Could you check a few things on this model? Use its own coordinates, in mm. A direction names the side the tool comes from. Give positions to 0.01 mm unless a question says otherwise; leave off trailing zeros. Loops run counter-clockwise (first coordinate to the right, second up) from the corner with the lowest first, then second, coordinate; pieces in that order, holes last. Notation, with made-up numbers: (89, -16) - (148, -16) arc R29 cw to (148, 8) - close; hole circle Ø4 at (-34.75, 31.5). An arc over 180 degrees is marked (long way). One line per item, written item: value. Start each with the question number.
Q1. I want a section at B-B (z = -75). Count the separate pieces of the cut face and the enclosed holes in it, then the cut area to 4 significant figures.
Q2. If I drill on line 1 (Z direction, x = -70, y = -0.85); line 2 (Z direction, x = 31, y = -1.4); line 3 (X direction, y = -1.8, z = 147.5), over which ranges is the centre line in solid material (lowest first)? Write a range as from..to.
Q3. For faces 5 (the face through (77.15, -0.04, 93.01)), 6 (the face through (-2, 2.5, -59)), which set-ups out of +Z, -Z, +X, -X, +Y, -Y let a thin tool reach every point of the face, with its end or its side?
Q4. If we mould it in two halves opening along Z, with no side actions, what happens to faces 1 (the face through (42.932, 0.035, -76.041)), 2 (the face through (-2, -2.5, -59)), 3 (the face through (-111.867, -0.035, -244.587)), 4 (the face through (-111.867, 0.035, 244.587))? For each: released by +Z, released by -Z, zero draft, split by the parting line, or undercut.
Q5. I want a section at A-A (z = 141). Please give me the cut outline in (x, y).
Q6. I'm going to push flat-ended pins straight in: P1, Ø3, axis at x = -35, z = 12, coming from the -Y side; P2, Ø4, axis at x = -35, z = -63, coming from the +Y side. Where does each tip first touch, or does it pass through?
```python
from build123d import *

# Parameters (mm, degrees)
SKETCH1_W            = 234
SKETCH1_H            = 500
BOSS_EXTRUDE1_DEPTH  = 2.5
M4_CLEARANCE_HOLE1_D = 4.8
FILLET1_R            = 18
M4_TAPPED_HOLE7_D    = 3.3
SKETCH4_R            = 14.75
SKETCH4_R_2          = 8
CUT_EXTRUDE6_DEPTH   = 277.068831997
M4_TAPPED_HOLE3_D    = 3.3
SKETCH9_R            = 14.75
CUT_EXTRUDE3_DEPTH   = 277.068831997
M4_TAPPED_HOLE4_D    = 3.3
SKETCH12_W           = 160
SKETCH12_H           = 120
CUT_EXTRUDE4_DEPTH   = 277.068831997
FILLET2_R            = 10


with BuildPart() as part:
    # Sketch1 → Boss-Extrude1 (new, symmetric)
    with BuildSketch(Plane(origin=(0, 0, 0), x_dir=(1, 0, 0), z_dir=(0, 1, 0))):
        Rectangle(SKETCH1_W, SKETCH1_H)
    extrude(amount=BOSS_EXTRUDE1_DEPTH, both=True)

    # M4 Clearance Hole1 (through all)
    with Locations(Plane(origin=(-75, 2.5, -242.5), x_dir=(0, 0, 1), z_dir=(0, 1, 0))):
        with Locations((0, 0), (0, 150), (67.5, 184.5), (67.5, -34.5), (242.5, 184.5), (242.5, -34.5), (417.5, -34.5), (417.5, 184.5), (485, 0), (485, 150)):
            Hole(M4_CLEARANCE_HOLE1_D / 2)

    # Fillet1
    fillet1_edges = [part.edges().sort_by_distance(p)[0] for p in [
        (117, 0, 250),
        (-117, 0, 250),
        (-117, 0, -250),
        (117, 0, -250),
    ]]
    fillet(fillet1_edges, radius=FILLET1_R)

    # M4 Tapped Hole7 (through all)
    with Locations(Plane(origin=(-85, 2.5, -87), x_dir=(0, 0, 1), z_dir=(0, 1, 0))):
        with Locations((0, 0), (24, 0), (24, 25), (0, 25), (0, 50), (24, 50), (-6, 85), (30, 85), (0, 120), (24, 120), (0, 145), (24, 145), (0, 170), (24, 170), (75, 120), (99, 120), (75, 50), (99, 50)):
            Hole(M4_TAPPED_HOLE7_D / 2)

    # Sketch4 → Cut-Extrude6 (cut, through all)
    with BuildSketch(Plane(origin=(0, 2.5, 0), x_dir=(1, 0, 0), z_dir=(0, 1, 0))):
        with Locations(Location((0, 75, 0), (0, 0, 270))):
            Circle(SKETCH4_R)
        with Locations(Location((-35, 75, 0), (0, 0, 270))):
            Circle(SKETCH4_R_2)
        with Locations(Location((35, 75, 0), (0, 0, 270))):
            Circle(SKETCH4_R_2)
        with Locations(Location((-60, 75, 0), (0, 0, 270))):
            Circle(SKETCH4_R_2)
        with Locations(Location((-85, 75, 0), (0, 0, 270))):
            Circle(SKETCH4_R_2)
        with Locations(Location((60, 75, 0), (0, 0, 270))):
            Circle(SKETCH4_R_2)
        with Locations(Location((85, 75, 0), (0, 0, 270))):
            Circle(SKETCH4_R_2)
        with Locations(Location((35, 0, 0), (0, 0, 270))):
            Circle(SKETCH4_R_2)
        with Locations(Location((-35, 0, 0), (0, 0, 270))):
            Circle(SKETCH4_R_2)
    extrude(amount=-CUT_EXTRUDE6_DEPTH, mode=Mode.SUBTRACT)

    # M4 Tapped Hole3 (through all)
    with Locations(Plane(origin=(0, 2.5, -18), x_dir=(0, 0, 1), z_dir=(0, 1, 0))):
        with Locations((0, 0), (36, 0)):
            Hole(M4_TAPPED_HOLE3_D / 2)

    # Sketch9 → Cut-Extrude3 (cut, through all)
    with BuildSketch(Plane(origin=(0, 2.5, 0), x_dir=(1, 0, 0), z_dir=(0, 1, 0))):
        with Locations(Location((0, 0, 0), (0, 0, 270))):
            Circle(SKETCH9_R)
    extrude(amount=-CUT_EXTRUDE3_DEPTH, mode=Mode.SUBTRACT)

    # M4 Tapped Hole4 (through all)
    with Locations(Plane(origin=(-70, 2.5, 80), x_dir=(0, 0, 1), z_dir=(0, 1, 0))):
        with Locations((0, 0), (0, 140), (140, 140), (140, 0)):
            Hole(M4_TAPPED_HOLE4_D / 2)

    # Sketch12 → Cut-Extrude4 (cut, through all)
    with BuildSketch(Plane(origin=(0, 2.5, 0), x_dir=(1, 0, 0), z_dir=(0, 1, 0))):
        with Locations((0, -150)):
            Rectangle(SKETCH12_W, SKETCH12_H)
    extrude(amount=-CUT_EXTRUDE4_DEPTH, mode=Mode.SUBTRACT)

    # Fillet2
    fillet2_edges = [part.edges().sort_by_distance(p)[0] for p in [
        (80, 0, 90),
        (80, 0, 210),
        (-80, 0, 210),
        (-80, 0, 90),
    ]]
    fillet(fillet2_edges, radius=FILLET2_R)


solid = part.part
```
Worked answers:
1. separate pieces: 8
1. enclosed holes: 0
1. area: 542.5 mm²
2. line 1: z = -250..78.35, 81.65..90, 210..218.35, 221.65..250
2. line 2: z = -250..-81.93, -68.07..-6.93, 6.93..90, 210..250
2. line 3: x = -117..-80, 80..117
3. face 5: +Y, -Y
3. face 6: +Z, -Z, +X, -X, +Y
4. face 1: undercut
4. face 2: zero draft
4. face 3: released by -Z
4. face 4: released by +Z
5. outline: (-117, -2.5) - (-80, -2.5) - (-80, 2.5) - (-117, 2.5) - close; (80, -2.5) - (117, -2.5) - (117, 2.5) - (80, 2.5) - close
6. P1: passes through
6. P2: stops at y = 2.5
